```python
from build123d import *

# Parameters (mm, degrees)
BOSS_EXTRUDE1_DEPTH = 500
CUT_EXTRUDE1_DEPTH  = 504.115294937


with BuildPart() as part:
    # Sketch1 → Boss-Extrude1 (new, symmetric)
    with BuildSketch(Plane.XY):
        with BuildLine():
            Line((-17, -25), (17, -25))
            ThreePointArc((17, -25), (22.656854249, -22.656854249), (25, -17))
            Line((25, -17), (25, 17))
            ThreePointArc((25, 17), (22.656854249, 22.656854249), (17, 25))
            Line((17, 25), (-17, 25))
            ThreePointArc((-17, 25), (-22.656854249, 22.656854249), (-25, 17))
            Line((-25, 17), (-25, -17))
            ThreePointArc((-25, -17), (-22.656854249, -22.656854249), (-17, -25))
        make_face()
        with BuildLine():
            Line((-17, 21), (17, 21))
            ThreePointArc((17, 21), (19.828427125, 19.828427125), (21, 17))
            Line((21, 17), (21, -17))
            ThreePointArc((21, -17), (19.828427125, -19.828427125), (17, -21))
            Line((17, -21), (-17, -21))
            ThreePointArc((-17, -21), (-19.828427125, -19.828427125), (-21, -17))
            Line((-21, -17), (-21, 17))
            ThreePointArc((-21, 17), (-19.828427125, 19.828427125), (-17, 21))
        make_face(mode=Mode.SUBTRACT)
    extrude(amount=BOSS_EXTRUDE1_DEPTH, both=True)

    # Sketch2 → Cut-Extrude1 (cut, through all)
    with BuildSketch(Plane.ZY.offset(25)):
        Polygon((-500, 25), (-450, -25), (-500, -25), align=None)
    cut_extrude1 = extrude(amount=-CUT_EXTRUDE1_DEPTH, mode=Mode.SUBTRACT)

    # Mirror1: Cut-Extrude1 across plane
    add(cut_extrude1.mirror(Plane.XY), mode=Mode.SUBTRACT)


solid = part.part
```
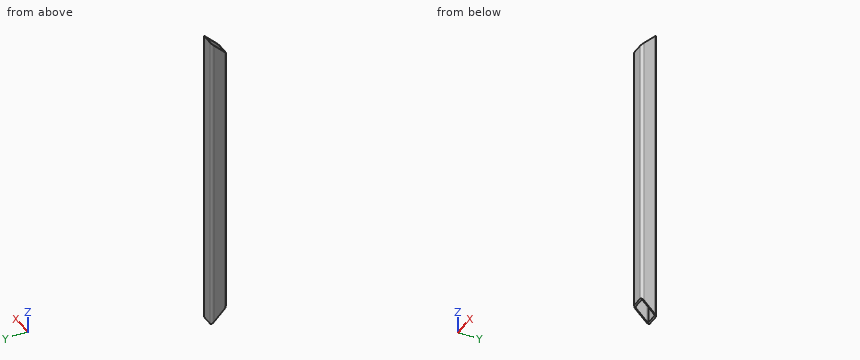
The listing builds one solid part. Answer for the finished solid, in the listing's coordinates (mm). Coordinates: 2 decimals unless noted, no trailing zeros. Loops run counter-clockwise (first coordinate to the right, second up) from the corner with the lowest first, then second, coordinate; pieces in that order, holes last. Notation, with made-up numbers: (37.5, -12) -> (50.5, -12) arc R15 ccw to (50.5, 11) -> close; hole circle Ø4 at (-4.5, 35). An arc over 180 degrees is marked (long way). Use one line per item in the form item = value. Start each with the question number.
Item 1: The part is cut by section C-C on z = 130. Determine the outline of the cut face in (x, y).
Item 2: The part is cut by section B-B on x = 5. Determine the outline of the cut face in (y, z), then the cut area to 3 significant figures.
Item 3: Consider L1, parallel to X at y = -12, z = -404; L2, parallel to Y at x = -18, z = -40.5. Determine where each line is inside the solid, lowest interval first. Write a range as [from, to].
Item 4: The part is cut by section A-A on y = 7.5. Determine the outline of the cut face in (x, z).
Answer key:
q1.outline = (-25, -17) arc R8 ccw to (-17, -25) -> (17, -25) arc R8 ccw to (25, -17) -> (25, 17) arc R8 ccw to (17, 25) -> (-17, 25) arc R8 ccw to (-25, 17) -> close; hole (-21, -17) arc R4 ccw to (-17, -21) -> (17, -21) arc R4 ccw to (21, -17) -> (21, 17) arc R4 ccw to (17, 21) -> (-17, 21) arc R4 ccw to (-21, 17) -> close
q2.outline = (-25, -450) -> (-21, -454) -> (-21, 454) -> (-25, 450) -> close; (21, -496) -> (25, -500) -> (25, 500) -> (21, 496) -> close
q2.area = 7,600 mm2
q3.L1 = [-25, -21], [21, 25]
q3.L2 = [-24.94, -20.87], [20.87, 24.94]
q4.outline = (-25, -482.5) -> (-21, -482.5) -> (-21, 482.5) -> (-25, 482.5) -> close; (21, -482.5) -> (25, -482.5) -> (25, 482.5) -> (21, 482.5) -> close
